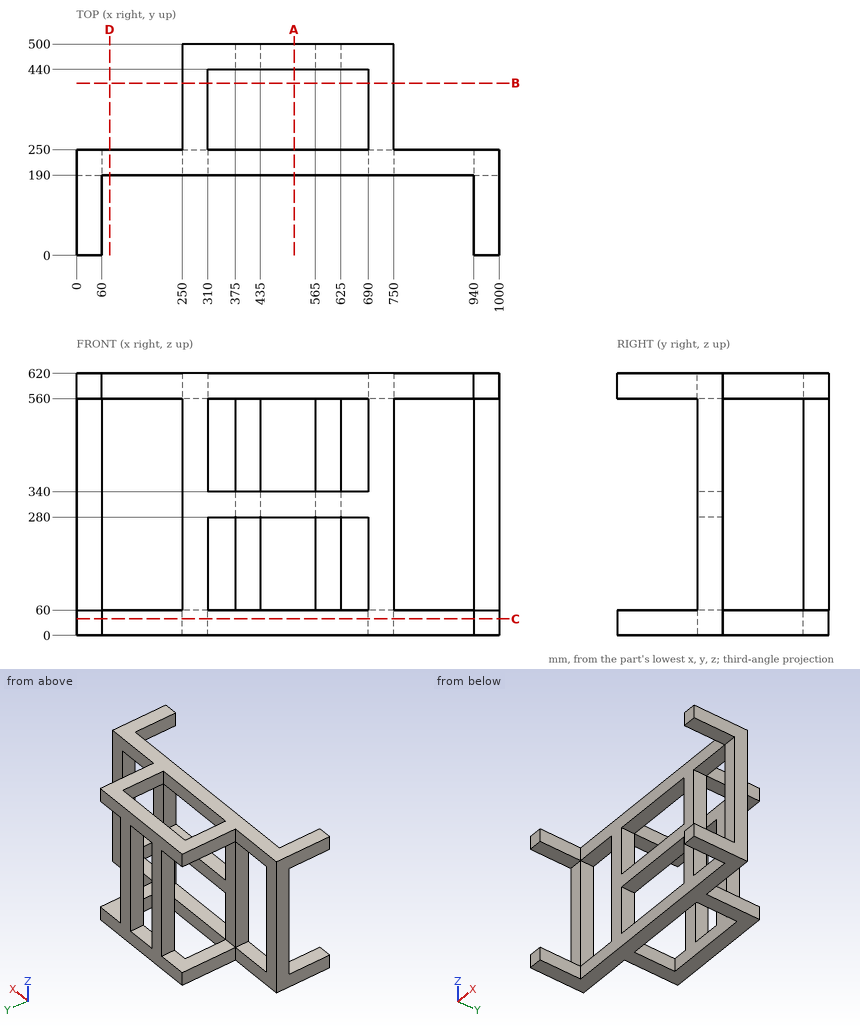
Check sheet for the drawn part. Datum: minimum x, y, z corner. Units: mm. Give positions to 0.01 mm unless a question says otherwise; leave off trailing zeros. Loops run counter-clockwise (first coordinate to the right, second up) from the corner with the lowest first, then second, coordinate; pieces in that order, holes last.
1) Thickness scan on line 1 along X through (y, z) = (228, 117.5); line 2 along Z through (x, y) = (702, 425.5); line 3 along X through (y, z) = (477, 205). Record the ranges inside material, lowest first.
2) Sectioned sample at C-C, the plane z = 39. Enter the section's corners in (x, y).
3) Sectioned sample at A-A, the plane x = 515. Enter the section's corners in (y, z), then the cut area to 3 significant figures.
4) Depth check by flat-ended pin: pin 1 Ø18 at (y, z) = (480, 421) entering from -X; pin 2 Ø3 at (x, z) = (316, 279) entering from +Y. Enter the tip coordinate at first touch or a pass-through.
5) Sectioned sample at B-B, the plane y = 407.5. Enter the section's corners in (x, z).
6) Sectioned sample at D-D, the plane x = 78.5. Enter the section's corners in (y, z), then the cut area to 3 significant figures.
Answers:
1. line 1: x = 0 to 60, 250 to 310, 690 to 750, 940 to 1000
1. line 2: z = 0 to 60, 560 to 620
1. line 3: x = 375 to 435, 565 to 625
2. outline: (0, 0) - (60, 0) - (60, 190) - (940, 190) - (940, 0) - (1000, 0) - (1000, 250) - (750, 250) - (750, 500) - (250, 500) - (250, 250) - (0, 250) - close; hole (310, 250) - (690, 250) - (690, 440) - (310, 440) - close
3. outline: (190, 0) - (250, 0) - (250, 60) - (190, 60) - close; (190, 280) - (250, 280) - (250, 340) - (190, 340) - close; (190, 560) - (250, 560) - (250, 620) - (190, 620) - close; (440, 0) - (500, 0) - (500, 60) - (440, 60) - close; (440, 560) - (500, 560) - (500, 620) - (440, 620) - close
3. area: 18,000 mm2
4. pin 1: stops at x = 375
4. pin 2: stops at y = 250
5. outline: (250, 0) - (310, 0) - (310, 60) - (250, 60) - close; (250, 560) - (310, 560) - (310, 620) - (250, 620) - close; (690, 0) - (750, 0) - (750, 60) - (690, 60) - close; (690, 560) - (750, 560) - (750, 620) - (690, 620) - close
6. outline: (190, 0) - (250, 0) - (250, 60) - (190, 60) - close; (190, 560) - (250, 560) - (250, 620) - (190, 620) - close
6. area: 7,200 mm2
